Source: CAD feature listing. Evaluate the final solid. Frame: model axes, mm. A direction names the side the tool comes from. Round coordinates to 2 decimals unless told otherwise and drop trailing zeros. Order: outer loops, then holes, each group sorted by start corner. A loop starts at its lowest first (then second) coordinate and runs counter-clockwise, first axis right, second up. Notation, with made-up numbers: (5, -0.5) - (62, -0.5) arc R7 ccw to (62, 9.5) - close; hole circle Ø4 at (63.25, 48). An arc over 180 degrees is marked (long way). Put each result on its own line as item: value. Start each with the question number.
1) Section A-A on x = 25. Output: boundary loops of the cut face in (y, z), then the cut area to 3 significant figures.
2) Contact query for flat-ended pins moving along their axis: P1, Ø1.5, axis at x = 19, y = -1, coming from the +Z side; P2, Ø3, axis at x = 9.5, z = 3.5, coming from the +Y side; P3, Ø5, axis at x = 20.5, z = 2, coming from the -Y side. Output: stop coordinate, or through.
3) Line query: probe 1 along X at (y, z) = (-1.5, 2.75); probe 2 along Y at (x, z) = (30, -2); probe 3 along Z at (x, y) = (32.5, -2.75). Output: solid intervals per line, ascending. Write a range as [from, to].
4) Access query for faces 1 (the face through (1.726, 4.31, -2.535)), 2 (the face through (4, -3, 1)). Directions: +Z, -Z, +X, -X, +Y, -Y. A direction counts if a zero-diameter tool reaches every point of the face in a straight line with its end or side. Return the directions, or none.
```python
from build123d import *

# Parameters (mm, degrees)
BASEHEAD_DEPTH = 4
SKETCH5_R      = 3
BASEBODY_DEPTH = 30
CHAMFER1_SIZE  = 0.3


with BuildPart() as part:
    # Sketch2 → BaseHead (new body)
    with BuildSketch(Plane(origin=(0, 0, 0), x_dir=(0, 0, -1), z_dir=(1, 0, 0))):
        Polygon((0, -5.773502692), (5, -2.886751346), (5, 2.886751346), (0, 5.773502692), (-5, 2.886751346), (-5, -2.886751346), align=None)
    extrude(amount=BASEHEAD_DEPTH)

    # Sketch3 → BearingFace (revolve, cut)
    with BuildSketch(Plane.XY, mode=Mode.PRIVATE) as bearingface_sk:
        Polygon((4, 5.773502692), (4, 4.37), (3.5, 4.87), (3.5, 5.773502692), align=None)
    revolve(bearingface_sk.sketch.rotate(Axis((-0.957090588, 0, 0), (1, 0, 0)), 90), axis=Axis((-0.957090588, 0, 0), (1, 0, 0)), mode=Mode.SUBTRACT)

    # Sketch4 → HeadChamfer (revolve, cut)
    with BuildSketch(Plane.XY):
        Polygon((0, 5.773502692), (0.281531956, 5.773502692), (0, 5), align=None)
    revolve(axis=Axis((-0.493528746, 0, 0), (1, 0, 0)), mode=Mode.SUBTRACT)

    # Sketch5 → BaseBody (add)
    with BuildSketch(Plane(origin=(4, 0, 0), x_dir=(0, 0, -1), z_dir=(1, 0, 0))):
        Circle(SKETCH5_R)
    extrude(amount=BASEBODY_DEPTH)

    # Chamfer1
    chamfer1_edges = [part.edges().sort_by_distance(p)[0] for p in [
        (34, 0, 3),
    ]]
    chamfer(chamfer1_edges, length=CHAMFER1_SIZE)


solid = part.part
```
Answer sheet:
1. outline: circle Ø6 at (0, 0)
1. area: 28.3 mm^2
2. P1: z = 2.99
2. P2: y = 2.24
2. P3: y = -3
3. probe 1: [0, 4]
3. probe 2: [-2.24, 2.24]
3. probe 3: [-1.2, 1.2]
4. face 1: -Z, +X, -X, +Y
4. face 2: +X
